Work out the finished part from the listing and answer in its coordinate system (mm). A direction names the side the tool comes from. Round coordinates to 2 decimals unless told otherwise and drop trailing zeros. Loops run counter-clockwise (first coordinate to the right, second up) from the corner with the lowest first, then second, coordinate; pieces in that order, holes last.
```python
from build123d import *
from OCP.BRepFilletAPI import BRepFilletAPI_MakeFillet

# Parameters (mm, degrees)
PLATE_AND_BOSS_PROFILE_W             = 154
PLATE_AND_BOSS_PROFILE_H             = 154
PLATE_AND_BOSS_PROFILE_R             = 18
BASE_PLATE_DEPTH                     = 25
CENTRAL_START                        = 25
SKETCH1_3_R                          = 18
CENTRAL_BOSS_AND_LUGS_DEPTH          = 31
PLATE_AND_BOSS_FILLETS_R26_R12_R1    = 12
PLATE_AND_BOSS_FILLETS_R26_R12_R2    = 26
LUG_PIN_HOLES_10_D                   = 10
LUG_PIN_HOLES_10_CSINK_D             = 10.05
LUG_PIN_HOLES_10_CSINK_ANGLE         = 90
LOCATING_SPIGOT_PROFILE_112_W        = 112
LOCATING_SPIGOT_PROFILE_112_H        = 112
LOCATING_SPIGOT_DEPTH                = 6
CENTRAL_BORE_28_CBORE_40_D           = 28
CENTRAL_BORE_28_CBORE_40_CBORE_D     = 40
CENTRAL_BORE_28_CBORE_40_CBORE_DEPTH = 42
PLATE_MOUNTING_HOLES_20_D            = 20
BOSS_TAPPED_HOLES_M22X2_0_D          = 20
BOSS_TAPPED_HOLES_M22X2_0_DEPTH      = 26
BOSS_TAPPED_HOLES_M22X2_0_TIP        = 6.00860619


with BuildPart() as part:
    # Plate and Boss Profile → Base Plate (new body)
    # profile 1 of 4: a face of its own
    with BuildSketch(Plane(origin=(0, 0, 0), x_dir=(1, 0, 0), z_dir=(0, 1, 0))):
        Rectangle(PLATE_AND_BOSS_PROFILE_W, PLATE_AND_BOSS_PROFILE_H)
        with BuildLine():
            Line((-26.719653956, 19), (-17.266235066, 51.086956522))
            ThreePointArc((-17.266235066, 51.086956522), (0, 64), (17.266235066, 51.086956522))
            Line((17.266235066, 51.086956522), (26.719653956, 19))
            Line((26.719653956, 19), (63, 19))
            Line((63, 19), (63, 9))
            Line((63, 9), (31, 9))
            Line((31, 9), (31, -9))
            Line((31, -9), (63, -9))
            Line((63, -9), (63, -19))
            Line((63, -19), (26.719653956, -19))
            Line((26.719653956, -19), (17.266235066, -51.086956522))
            ThreePointArc((17.266235066, -51.086956522), (0, -64), (-17.266235066, -51.086956522))
            Line((-17.266235066, -51.086956522), (-26.719653956, -19))
            Line((-26.719653956, -19), (-63, -19))
            Line((-63, -19), (-63, -9))
            Line((-63, -9), (-31, -9))
            Line((-31, -9), (-31, 9))
            Line((-31, 9), (-63, 9))
            Line((-63, 9), (-63, 19))
            Line((-63, 19), (-26.719653956, 19))
        make_face(mode=Mode.SUBTRACT)
    # profile 2 of 4: a face of its own
    with BuildSketch(Plane(origin=(0, 0, 0), x_dir=(1, 0, 0), z_dir=(0, 1, 0))):
        with BuildLine():
            ThreePointArc((18, 46), (-2.569802406, 28.184385624), (-17.266235066, 51.086956522))
            Line((-17.266235066, 51.086956522), (-26.719653956, 19))
            Line((-26.719653956, 19), (-63, 19))
            Line((-63, 19), (-63, 9))
            Line((-63, 9), (-31, 9))
            Line((-31, 9), (-31, -9))
            Line((-31, -9), (-63, -9))
            Line((-63, -9), (-63, -19))
            Line((-63, -19), (-26.719653956, -19))
            Line((-26.719653956, -19), (-17.266235066, -51.086956522))
            ThreePointArc((-17.266235066, -51.086956522), (-2.569802406, -28.184385624), (18, -46))
            ThreePointArc((18, -46), (17.815614376, -48.569802406), (17.266235066, -51.086956522))
            Line((17.266235066, -51.086956522), (26.719653956, -19))
            Line((26.719653956, -19), (63, -19))
            Line((63, -19), (63, -9))
            Line((63, -9), (31, -9))
            Line((31, -9), (31, 9))
            Line((31, 9), (63, 9))
            Line((63, 9), (63, 19))
            Line((63, 19), (26.719653956, 19))
            Line((26.719653956, 19), (17.266235066, 51.086956522))
            ThreePointArc((17.266235066, 51.086956522), (17.815614376, 48.569802406), (18, 46))
        make_face()
    # profile 3 of 4: a face of its own
    with BuildSketch(Plane(origin=(0, 0, 0), x_dir=(1, 0, 0), z_dir=(0, 1, 0))):
        with Locations((0, 46)):
            Circle(PLATE_AND_BOSS_PROFILE_R)
    # profile 4 of 4: a face of its own
    with BuildSketch(Plane(origin=(0, 0, 0), x_dir=(1, 0, 0), z_dir=(0, 1, 0))):
        with Locations((0, -46)):
            Circle(PLATE_AND_BOSS_PROFILE_R)
    extrude(amount=BASE_PLATE_DEPTH)

    # Sketch1_3 → Central Boss and Lugs (add)
    with BuildSketch(Plane(origin=(0, 0, 0), x_dir=(1, 0, 0), z_dir=(0, 1, 0)).offset(CENTRAL_START)):
        with BuildLine():
            ThreePointArc((18, 46), (-2.569802406, 28.184385624), (-17.266235066, 51.086956522))
            Line((-17.266235066, 51.086956522), (-26.719653956, 19))
            Line((-26.719653956, 19), (-63, 19))
            Line((-63, 19), (-63, 9))
            Line((-63, 9), (-31, 9))
            Line((-31, 9), (-31, -9))
            Line((-31, -9), (-63, -9))
            Line((-63, -9), (-63, -19))
            Line((-63, -19), (-26.719653956, -19))
            Line((-26.719653956, -19), (-17.266235066, -51.086956522))
            ThreePointArc((-17.266235066, -51.086956522), (-2.569802406, -28.184385624), (18, -46))
            ThreePointArc((18, -46), (17.815614376, -48.569802406), (17.266235066, -51.086956522))
            Line((17.266235066, -51.086956522), (26.719653956, -19))
            Line((26.719653956, -19), (63, -19))
            Line((63, -19), (63, -9))
            Line((63, -9), (31, -9))
            Line((31, -9), (31, 9))
            Line((31, 9), (63, 9))
            Line((63, 9), (63, 19))
            Line((63, 19), (26.719653956, 19))
            Line((26.719653956, 19), (17.266235066, 51.086956522))
            ThreePointArc((17.266235066, 51.086956522), (17.815614376, 48.569802406), (18, 46))
        make_face()
        with Locations((0, 46)):
            Circle(SKETCH1_3_R)
        with Locations((0, -46)):
            Circle(SKETCH1_3_R)
    extrude(amount=CENTRAL_BOSS_AND_LUGS_DEPTH)

    # Plate and Boss Fillets R26 R12: one fillet with a radius per group of edges: ONE call of the kernel's fillet builder (fillet() takes one radius for all edges)
    plate_and_boss_fillets_r26_r12_edges_1 = [part.edges().sort_by_distance(p)[0] for p in [
        (63, 56, 14),
        (-63, 56, -14),
        (63, 56, -14),
        (-63, 56, 14),
    ]]
    plate_and_boss_fillets_r26_r12_edges_2 = [part.edges().sort_by_distance(p)[0] for p in [
        (77, 12.5, 77),
        (-77, 12.5, 77),
        (-77, 12.5, -77),
        (77, 12.5, -77),
    ]]
    plate_and_boss_fillets_r26_r12 = BRepFilletAPI_MakeFillet(part.part.solid().wrapped)
    for e in plate_and_boss_fillets_r26_r12_edges_1:
        plate_and_boss_fillets_r26_r12.Add(PLATE_AND_BOSS_FILLETS_R26_R12_R1, e.wrapped)
    for e in plate_and_boss_fillets_r26_r12_edges_2:
        plate_and_boss_fillets_r26_r12.Add(PLATE_AND_BOSS_FILLETS_R26_R12_R2, e.wrapped)
    add(Compound.cast(plate_and_boss_fillets_r26_r12.Shape()), mode=Mode.REPLACE)

    # Lug Pin Holes _10 (through all)
    with Locations(Plane.XY.offset(19)):
        with Locations((-51, 44), (51, 44)):
            CounterSinkHole(LUG_PIN_HOLES_10_D / 2, LUG_PIN_HOLES_10_CSINK_D / 2, counter_sink_angle=LUG_PIN_HOLES_10_CSINK_ANGLE)

    # Locating Spigot Profile _112 → Locating Spigot (add)
    with BuildSketch(Plane.XZ):
        Rectangle(LOCATING_SPIGOT_PROFILE_112_W, LOCATING_SPIGOT_PROFILE_112_H)
    extrude(amount=LOCATING_SPIGOT_DEPTH)

    # Central Bore _28 Cbore _40 (through all)
    with Locations(Plane(origin=(0, 56, 0), x_dir=(1, 0, 0), z_dir=(0, 1, 0))):
        with Locations((0, 0)):
            CounterBoreHole(CENTRAL_BORE_28_CBORE_40_D / 2, CENTRAL_BORE_28_CBORE_40_CBORE_D / 2, CENTRAL_BORE_28_CBORE_40_CBORE_DEPTH)

    # Plate Mounting Holes _20 (through all)
    with Locations(Plane(origin=(0, 25, 0), x_dir=(1, 0, 0), z_dir=(0, 1, 0))):
        with Locations((51, -51), (51, 51), (-51, 51), (-51, -51)):
            Hole(PLATE_MOUNTING_HOLES_20_D / 2)

    # Boss Tapped Holes M22x2.0
    with Locations(Plane(origin=(0, 56, 0), x_dir=(1, 0, 0), z_dir=(0, 1, 0))):
        with Locations((0, -46), (0, 46)):
            Hole(BOSS_TAPPED_HOLES_M22X2_0_D / 2, depth=BOSS_TAPPED_HOLES_M22X2_0_DEPTH)
            with Locations((0, 0, -(BOSS_TAPPED_HOLES_M22X2_0_DEPTH + BOSS_TAPPED_HOLES_M22X2_0_TIP / 2))):  # 118° drill point
                Cone(0, BOSS_TAPPED_HOLES_M22X2_0_D / 2, BOSS_TAPPED_HOLES_M22X2_0_TIP, mode=Mode.SUBTRACT)


solid = part.part
```
1. Find section B-B (z = 22). Write down the section's boundary in (x, y).
Answer key:
outline: (-77, 0) - (-56, 0) - (-56, -6) - (56, -6) - (56, 0) - (77, 0) - (77, 25) - (25.84, 25) - (25.84, 56) - (-25.84, 56) - (-25.84, 25) - (-77, 25) - close
2. Consider probe 1 along Z at (x, y) = (51, 9); probe 2 along X at (y, z) = (7, 1); probe 3 along Z at (x, y) = (59, 29). Determine where each line is inside the solid, lowest interval first.
Answer key:
probe 1: z = -77 to -61, -41 to 41, 61 to 77
probe 2: x = -77 to -13.96, 13.96 to 77
probe 3: z = -19 to -9, 9 to 19
3. Find section A-A (y = 32.5). Write down the section's boundary in (x, z), then the cut area to 3 significant figures.
Answer key:
outline: (-63, -19) - (-26.72, -19) - (-17.27, -51.09) arc R18 ccw to (17.27, -51.09) - (26.72, -19) - (63, -19) - (63, -9) - (31, -9) - (31, 9) - (63, 9) - (63, 19) - (26.72, 19) - (17.27, 51.09) arc R18 ccw to (-17.27, 51.09) - (-26.72, 19) - (-63, 19) - (-63, 9) - (-31, 9) - (-31, -9) - (-63, -9) - close; hole circle Ø40 at (0, 0); hole circle Ø20 at (0, -46); hole circle Ø20 at (0, 46)
area: 5,230 mm2
4. Which of the six approach directions +Z, -Z, +X, -X, +Y, -Y give full straight-line access (tool end or side, diameter ignored) to faces 1 (the face through (33, 25, -1)), 2 (the face through (-21.927, 40.283, -35.268)), 3 (the face through (0, 40, -64))?
Answer key:
face 1: +Y
face 2: -Z, -X, +Y
face 3: -Z, +Y
5. Determine the mould class of faces 4 (the face through (-13, -6, 13)), 5 (the face through (-50.349, 48.957, 13.918)), 6 (the face through (63, 34, -14)), 7 (the face through (0.93, 25.03, -47.46)) for opening direction X: +X half, -X half, draft (parallel to the pull), parting line (faces both ways), or undercut.
Answer key:
face 4: draft
face 5: undercut
face 6: +X half
face 7: undercut
6. Given pin 1 (5 mm diameter, centred on y = 38.5, z = -44, fed in from -X); pin 2 (12 mm diameter, centred on y = 36.5, z = -18.5, fed in from -X); pin 3 (9.5 mm diameter, centred on x = 42, y = 47, fed in from -Z); pin 4 (6.5 mm diameter, centred on x = -0.5, y = -3, fed in from -Z), each flat-ended and moving along its own axis, determine where each tip first touches the part or whether it passes through.
Answer key:
pin 1: stops at x = -20.09
pin 2: stops at x = -63
pin 3: stops at z = -19
pin 4: stops at z = -77
